Input: part model. Units: mm. Frame: model coordinates. Coordinates: 2 decimals unless noted, no trailing zeros. Loops run counter-clockwise (first coordinate to the right, second up) from the corner with the lowest first, then second, coordinate; pieces in that order, holes last. Notation, with made-up numbers: M -15.5,-21.75 L 9.5,-21.75 A23 cw 9.5,-2.75 Z; hole C -32,35 d9. An arc over 180 degrees is marked long. Use a Markdown table: item, result. Add a question column.
1. Section A-A on z = 2.5. Output: boundary loops of the cut face in (x, y) (3 decimals), then the cut area to 3 significant figures.
2. Section C-C on y = -26.5. Output: boundary loops of the cut face in (x, z), then the cut area to 3 significant figures.
3. Draft query along Y for faces 1 (the flat face through (0, -14, 0)), 2 (the flat face through (0, 0, 4)), 3 (the cylindrical face through (0.45, -9.15, 5.07)). Return one class per face: +Y half, -Y half, draft (parallel to the pull), parting line (faces both ways), or undercut.
4. Section D-D on z = 9.5. Output: boundary loops of the cut face in (x, y) (3 decimals), then the cut area to 3 significant figures.
5. Line query: L1, parallel to Z at x = 0, y = -37.5; L2, parallel to Z at x = -0.5, y = -36; L3, parallel to X at y = -44, z = 3. Output: solid intervals per line, ascending. Write a range as [from, to].
6. Pin query (flat end, axial travel): pin 1 (1.5 mm diameter, centred on y = -32, z = 1.5, fed in from -X); pin 2 (3 mm diameter, centred on y = -42, z = 8.5, fed in from -X). Return the tip coordinate at first contact, or that it passes through.
7. Section B-B on z = 5.75. Output: boundary loops of the cut face in (x, y) (3 decimals).
```python
from build123d import *

# Parameters (mm, degrees)
EXTRUDE_1_DEPTH          = 10
SKETCH_3_R               = 0.975
CUT_EXTRUDE_2_DEPTH      = 61.959002617
FILLET_1_R               = 1.5
CUT_EXTRUDE_3_DEPTH      = 62.351446601
CUT_EXTRUDE_3_DEPTH_BACK = 62.351446601
SKETCH_6_R               = 12.5


with BuildPart() as part:
    # 草图1 → 凸台-拉伸1 (new body)
    with BuildSketch(Plane.XY):
        Polygon((-4, 0), (4, 0), (4, -25), (0, -60), (-4, -25), align=None)
    extrude(amount=EXTRUDE_1_DEPTH)

    # 草图3 → 切除-拉伸2 (cut, through all)
    with BuildSketch(Plane.XY.offset(10)):
        with Locations((0, -8.284315822)):
            Circle(SKETCH_3_R)
        with Locations((0, -2.584315822)):
            Circle(SKETCH_3_R)
    extrude(amount=-CUT_EXTRUDE_2_DEPTH, mode=Mode.SUBTRACT)

    # 圆角1
    fillet_1_edges = [part.edges().sort_by_distance(p)[0] for p in [
        (0, 0, 10),
    ]]
    fillet(fillet_1_edges, radius=FILLET_1_R)

    # 草图6 → 切除-拉伸3 (cut, two sides: drawn at the far end of the back side and taken through both)
    with BuildSketch(Plane.ZY.offset(4).offset(-CUT_EXTRUDE_3_DEPTH_BACK)):
        with Locations((-8.77, -37.5)):
            Circle(SKETCH_6_R)
    extrude(amount=CUT_EXTRUDE_3_DEPTH + CUT_EXTRUDE_3_DEPTH_BACK, mode=Mode.SUBTRACT)


solid = part.part
```
Answers below:
| question | item | result |
|---|---|---|
| 1 | outline | M -4,-25 L -3.189,-32.093 L 3.189,-32.093 L 4,-25 L 4,0 L -4,0 Z; M -1.953,-42.907 L 0,-60 L 1.953,-42.907 Z; hole C 0,-8.284 d1.95; hole C 0,-2.584 d1.95 |
| 1 | area | 278 mm² |
| 2 | outline | M -3.83,0 L 3.83,0 L 3.83,10 L -3.83,10 Z |
| 2 | area | 76.6 mm² |
| 3 | face 1 | draft |
| 3 | face 2 | +Y half |
| 3 | face 3 | undercut |
| 4 | outline | M -4,-25 L 0,-60 L 4,-25 L 4,-0.382 L -4,-0.382 Z; hole C 0,-8.284 d1.95; hole C 0,-2.584 d1.95 |
| 4 | area | 331 mm² |
| 5 | L1 | z = [3.73, 10] |
| 5 | L2 | z = [3.64, 10] |
| 5 | L3 | x = [-1.83, 1.83] |
| 6 | pin 1 | passes through |
| 6 | pin 2 | stops at x = -2.23 |
| 7 | outline | M -4,-25 L 0,-60 L 4,-25 L 4,0 L -4,0 Z; hole C 0,-8.284 d1.95; hole C 0,-2.584 d1.95 |
